Could you check a few things on this model? Use its own coordinates, in mm. A direction names the side the tool comes from. Coordinates: 2 decimals unless noted, no trailing zeros. Order: outer loops, then holes, each group sorted by start corner. A loop starts at its lowest first (then second) coordinate and runs counter-clockwise, first axis right, second up. Notation, with made-up numbers: (52.5, -19) - (59.5, -19) arc R15 cw to (59.5, -11) - close; hole circle Ø6 at (45, 83). An arc over 180 degrees is marked (long way). Answer as a JSON object with one key per item and string values. Group by question number.
(1) Imagine slicing it at B-B, the plane z = 0. Write out the boundary of the cut face in (x, y).
(2) Please list where these lines run through material, in increasing order: probe 1 along Y at (x, z) = (0.5, -68); probe 2 along Y at (x, z) = (89.5, -86.5); probe 3 along Z at (x, y) = (-89, 216.5).
(3) Imagine slicing it at C-C, the plane y = 261.5. Write out the boundary of the cut face in (x, z).
(4) Imagine slicing it at A-A, the plane x = 0. Write out the boundary of the cut face in (y, z), and give its area (3 significant figures).
(5) We'd pull the mould along Z, two halves only. Please class faces 1 (the flat face through (-1, 149, -100)), 2 (the cylindrical face through (3.604, 324.65, 11.446)), 3 (the cylindrical face through (28.836, 148.04, 91.567)), 4 (the flat face through (1, 0, -1)): pulls with the +Z half, pulls with the -Z half, needs draft (parallel to the pull), parting line crosses it, or undercut.
(6) Which directions (+Z, -Z, +X, -X, +Y, -Y) give clear straight access to the entire face, cutting with the end or side of a thin tool? Please do faces 5 (the flat face through (-86.932, 149.02, -80.167)), 6 (the flat face through (1, 80, -98)), 7 (the flat face through (1, 220, -98)).
(7) Will these pins go through, and if not, where does the flat tip stop? P1, Ø1, axis at y = 203, z = 28.5, coming from the -X side; P2, Ø1, axis at x = -80, z = -14.5, coming from the +Y side; P3, Ø10, axis at y = 173, z = 40, coming from the +X side.
(8) Imagine slicing it at D-D, the plane y = 191. Write out the boundary of the cut face in (x, z), and give its area (3 significant figures).
from build123d import *

# Parameters (mm, degrees)
SKETCH1_R           = 96
BOSS_EXTRUDE1_DEPTH = 300
SKETCH2_R           = 12
BOSS_EXTRUDE2_DEPTH = 50
FILLET1_R           = 10
BOSS_EXTRUDE3_DEPTH = 140


with BuildPart() as part:
    # Sketch1 → Boss-Extrude1 (new body)
    with BuildSketch(Plane(origin=(0, 0, 0), x_dir=(1, 0, 0), z_dir=(0, 1, 0))):
        with Locations(Location((0, 0, 0), (0, 0, 270))):
            Circle(SKETCH1_R)
    extrude(amount=BOSS_EXTRUDE1_DEPTH)

    # Sketch2 → Boss-Extrude2 (add)
    with BuildSketch(Plane(origin=(0, 300, 0), x_dir=(1, 0, 0), z_dir=(0, 1, 0))):
        with Locations(Location((0, 0, 0), (0, 0, 270))):
            Circle(SKETCH2_R)
    extrude(amount=BOSS_EXTRUDE2_DEPTH)

    # Fillet1
    fillet1_edges = [part.edges().sort_by_distance(p)[0] for p in [
        (0, 0, -96),
        (0, 300, -96),
    ]]
    fillet(fillet1_edges, radius=FILLET1_R)

    # Sketch3 → Boss-Extrude3 (add)
    with BuildSketch(Plane(origin=(0, 80, 0), x_dir=(-1, 0, 0), z_dir=(0, -1, 0))):
        with BuildLine():
            Line((74.225483886, 60.881668357), (100, 100))
            Line((100, 100), (-100, 100))
            Line((-100, 100), (-74.225483886, 60.881668357))
            ThreePointArc((-74.225483886, 60.881668357), (0, 96), (74.225483886, 60.881668357))
        make_face()
    extrude(amount=-BOSS_EXTRUDE3_DEPTH)


solid = part.part
Result set:
{
 "1": {"outline": "(-96, 10) arc R10 ccw to (-86, 0) - (86, 0) arc R10 ccw to (96, 10) - (96, 290) arc R10 ccw to (86, 300) - (12, 300) - (12, 350) - (-12, 350) - (-12, 300) - (-86, 300) arc R10 ccw to (-96, 290) - close"},
 "2": {"probe 1": "y = 0 to 300", "probe 2": "y = 80 to 220", "probe 3": "z = -100 to -83.31, -35.99 to 35.99"},
 "3": {"outline": "circle Ø192 at (0, 0)"},
 "4": {"outline": "(0, -86) arc R10 ccw to (10, -96) - (80, -96) - (80, -100) - (220, -100) - (220, -96) - (290, -96) arc R10 ccw to (300, -86) - (300, -12) - (350, -12) - (350, 12) - (300, 12) - (300, 86) arc R10 ccw to (290, 96) - (10, 96) arc R10 ccw to (0, 86) - close", "area": "59,300 mm^2"},
 "5": {"face 1": "pulls with the -Z half", "face 2": "parting line crosses it", "face 3": "undercut", "face 4": "needs draft"},
 "6": {"face 5": "-X, +Y, -Y", "face 6": "-Z, -Y", "face 7": "-Z, +Y"},
 "7": {"P1": "stops at x = -91.83", "P2": "stops at y = 300", "P3": "stops at x = 89.39"},
 "8": {"outline": "(-100, -100) - (100, -100) - (74.23, -60.88) arc R96 ccw (long way) to (-74.23, -60.88) - close", "area": "32,100 mm^2"}
}
